```python
from build123d import *

# Parameters (mm, degrees)
SKETCH_1_W                = 100
SKETCH_1_H                = 30
EXTRUDE_1_DEPTH           = 30
HOLE_WIZARD_1_D           = 9
HOLE_WIZARD_1_CBORE_D     = 15
HOLE_WIZARD_1_CBORE_DEPTH = 20
HOLE_WIZARD_M10_1_D       = 8.5


with BuildPart() as part:
    # 草图1 → 凸台-拉伸1 (new body)
    with BuildSketch(Plane.XY):
        Rectangle(SKETCH_1_W, SKETCH_1_H)
    extrude(amount=EXTRUDE_1_DEPTH)

    # 打孔尺寸(%根据)内六角圆柱头螺钉的类型1 (through all)
    with Locations(Plane(origin=(0, 15, 0), x_dir=(1, 0, 0), z_dir=(0, 1, 0))):
        with Locations((-35, -15), (35, -15)):
            CounterBoreHole(HOLE_WIZARD_1_D / 2, HOLE_WIZARD_1_CBORE_D / 2, HOLE_WIZARD_1_CBORE_DEPTH)

    # M10 螺纹孔1 (through all)
    with Locations(Plane.XY.offset(30)):
        with Locations((-20, 5), (20, 5)):
            Hole(HOLE_WIZARD_M10_1_D / 2)


solid = part.part
```
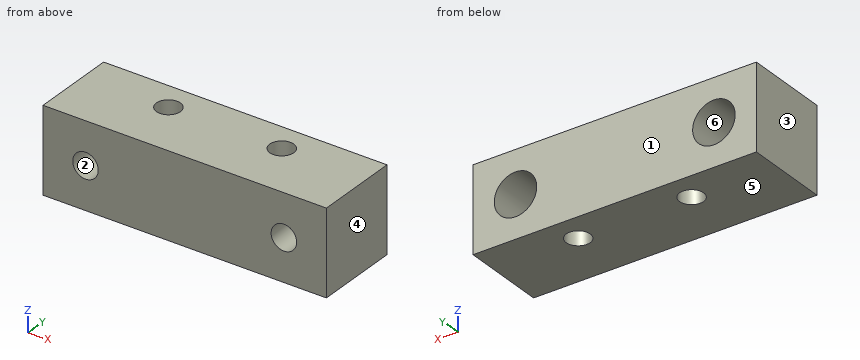
Geometry: final body of the model. Coordinates: model frame, mm. Face numbers are marked on the shaded views. A direction names the side the tool comes from. Coordinates: 2 decimals unless noted, no trailing zeros. Order: outer loops, then holes, each group sorted by start corner. A loop starts at its lowest first (then second) coordinate and runs counter-clockwise, first axis right, second up. Notation, with made-up numbers: M 40,52.5 L 46,52.5 A13 cw 46,67.5 Z; hole C 83.5,33.5 d10. An arc over 180 degrees is marked long. Answer in a Markdown table with one row per item. Add a question column.
Q1. Section query C-C on z = 14. Return the cut outline in (x, y).
Q2. Contact query for a flat-ended pin moving along its axis: P1, Ø4.5, axis at x = -33, z = 17, coming from the +Y side. Output: stop coordinate, or through.
Q3. Line query: L1, parallel to X at y = -6.75, z = 14.75; L2, parallel to Y at x = -20, z = 8.25; L3, parallel to Z at x = -35, y = -10.5. Output: solid intervals per line, ascending.
Q4. Section query A-A on y = 5. Return the cut outline in (x, z), and give its area (3 significant figures).
Q5. Section query D-D on y = -7.5. Return the cut outline in (x, z), and give its area (3 significant figures).
Q6. Mould query, pull axis X, two halves, no side actions, for the marked faces 1, 2, 3 and 4. Classes: released by +X, released by -X, zero draft, split by the parting line, or undercut.
Q7. Section query B-B on x = -35. Return the cut outline in (y, z), and give its area (3 significant figures).
Q8. Reachability of the marked faces 5 and 6 from +Z, -Z, +X, -X, +Y, -Y: full face, straight path, thin tool, end or side. Return the list, or none.
Completed:
| question | item | result |
|---|---|---|
| 1 | outline | M -50,-15 L -39.39,-15 L -39.39,-5 L -42.43,-5 L -42.43,15 L -50,15 Z; M -30.61,-15 L 30.61,-15 L 30.61,-5 L 27.57,-5 L 27.57,15 L -27.57,15 L -27.57,-5 L -30.61,-5 Z; M 39.39,-15 L 50,-15 L 50,15 L 42.43,15 L 42.43,-5 L 39.39,-5 Z; hole C -20,5 d8.5; hole C 20,5 d8.5 |
| 2 | P1 | stops at y = -5 |
| 3 | L1 | x = -50 to -39.49, -30.51 to 30.51, 39.49 to 50 |
| 3 | L2 | y = -15 to 0.75, 9.25 to 15 |
| 3 | L3 | z = 0 to 10.5, 19.5 to 30 |
| 4 | outline | M -50,0 L -24.25,0 L -24.25,30 L -50,30 Z; M -15.75,0 L 15.75,0 L 15.75,30 L -15.75,30 Z; M 24.25,0 L 50,0 L 50,30 L 24.25,30 Z; hole C -35,15 d15; hole C 35,15 d15 |
| 4 | area | 2,140 mm2 |
| 5 | outline | M -50,0 L 50,0 L 50,30 L -50,30 Z; hole C -35,15 d9; hole C 35,15 d9 |
| 5 | area | 2,870 mm2 |
| 6 | face 1 | zero draft |
| 6 | face 2 | undercut |
| 6 | face 3 | released by -X |
| 6 | face 4 | released by +X |
| 7 | outline | M -15,0 L 15,0 L 15,7.5 L -5,7.5 L -5,10.5 L -15,10.5 Z; M -15,19.5 L -5,19.5 L -5,22.5 L 15,22.5 L 15,30 L -15,30 Z |
| 7 | area | 510 mm2 |
| 8 | face 5 | -Z, +X, -X, +Y, -Y |
| 8 | face 6 | +Y |
